```python
from build123d import *

# Parameters (mm, degrees)
PLATE_OUTLINE_SKETCH_R = 10
BASE_PLATE_30MM_DEPTH  = 30
TOP_POCKET_CUT_DEPTH   = 25


with BuildPart() as part:
    # Plate Outline Sketch → Base Plate 30mm (new body)
    with BuildSketch(Plane(origin=(0, 0, 0), x_dir=(1, 0, 0), z_dir=(0, 1, 0))):
        with BuildLine():
            Line((-90, -88), (-90, -17.408786158))
            ThreePointArc((-90, -17.408786158), (-85.756556041, -5.090874739), (-74.826905826, 2))
            Line((-74.826905826, 2), (-4.826905826, 19.408786158))
            ThreePointArc((-4.826905826, 19.408786158), (0, 20), (4.826905826, 19.408786158))
            Line((4.826905826, 19.408786158), (74.826905826, 2))
            ThreePointArc((74.826905826, 2), (85.756556041, -5.090874739), (90, -17.408786158))
            Line((90, -17.408786158), (90, -88))
            ThreePointArc((90, -88), (78.164965809, -106.257418584), (56.666666667, -102.90711985))
            ThreePointArc((56.666666667, -102.90711985), (0, -81.262379212), (-56.666666667, -102.90711985))
            ThreePointArc((-56.666666667, -102.90711985), (-78.164965809, -106.257418584), (-90, -88))
        make_face()
        with Locations(Location((0, 0, 0), (0, 0, 270))):
            Circle(PLATE_OUTLINE_SKETCH_R, mode=Mode.SUBTRACT)
        with Locations(Location((-70, -88, 0), (0, 0, 270))):
            Circle(PLATE_OUTLINE_SKETCH_R, mode=Mode.SUBTRACT)
        with Locations(Location((70, -88, 0), (0, 0, 90))):
            Circle(PLATE_OUTLINE_SKETCH_R, mode=Mode.SUBTRACT)
        with BuildLine():
            Line((-80, -68.635083269), (-80, -17.408786158))
            ThreePointArc((-80, -17.408786158), (-75.428711332, -4.682637227), (-63.804513336, 2.226021665))
            Line((-63.804513336, 2.226021665), (-20.095749168, 10.695194253))
            ThreePointArc((-20.095749168, 10.695194253), (-15.433233379, 9.136955423), (-14.358465626, 4.339869223))
            ThreePointArc((-14.358465626, 4.339869223), (0, -15), (14.358465626, 4.339869223))
            ThreePointArc((14.358465626, 4.339869223), (15.433233379, 9.136955423), (20.095749168, 10.695194253))
            Line((20.095749168, 10.695194253), (63.804513336, 2.226021665))
            ThreePointArc((63.804513336, 2.226021665), (75.428711332, -4.682637227), (80, -17.408786158))
            Line((80, -17.408786158), (80, -68.635083269))
            ThreePointArc((80, -68.635083269), (78.061862178, -72.587930344), (73.75, -73.476312452))
            ThreePointArc((73.75, -73.476312452), (60.955053625, -76.033841674), (55.004181334, -87.645849573))
            ThreePointArc((55.004181334, -87.645849573), (52.221345421, -92.010026772), (47.064070693, -91.571010006))
            ThreePointArc((47.064070693, -91.571010006), (0, -76.262379212), (-47.064070693, -91.571010006))
            ThreePointArc((-47.064070693, -91.571010006), (-52.221345421, -92.010026772), (-55.004181334, -87.645849573))
            ThreePointArc((-55.004181334, -87.645849573), (-60.955053625, -76.033841674), (-73.75, -73.476312452))
            ThreePointArc((-73.75, -73.476312452), (-78.061862178, -72.587930344), (-80, -68.635083269))
        make_face(mode=Mode.SUBTRACT)
    extrude(amount=BASE_PLATE_30MM_DEPTH)

    # Top Pocket Sketch → Top Pocket Cut (add)
    with BuildSketch(Plane.XZ):
        with BuildLine():
            Line((-20.095749168, -10.695194253), (-63.804513336, -2.226021665))
            ThreePointArc((-63.804513336, -2.226021665), (-75.428711332, 4.682637227), (-80, 17.408786158))
            Line((-80, 17.408786158), (-80, 68.635083269))
            ThreePointArc((-80, 68.635083269), (-78.061862178, 72.587930344), (-73.75, 73.476312452))
            ThreePointArc((-73.75, 73.476312452), (-60.955053625, 76.033841674), (-55.004181334, 87.645849573))
            ThreePointArc((-55.004181334, 87.645849573), (-52.221345421, 92.010026772), (-47.064070693, 91.571010006))
            ThreePointArc((-47.064070693, 91.571010006), (0, 76.262379212), (47.064070693, 91.571010006))
            ThreePointArc((47.064070693, 91.571010006), (52.221345421, 92.010026772), (55.004181334, 87.645849573))
            ThreePointArc((55.004181334, 87.645849573), (60.955053625, 76.033841674), (73.75, 73.476312452))
            ThreePointArc((73.75, 73.476312452), (78.061862178, 72.587930344), (80, 68.635083269))
            Line((80, 68.635083269), (80, 17.408786158))
            ThreePointArc((80, 17.408786158), (75.428711332, 4.682637227), (63.804513336, -2.226021665))
            Line((63.804513336, -2.226021665), (20.095749168, -10.695194253))
            ThreePointArc((20.095749168, -10.695194253), (15.433233379, -9.136955423), (14.358465626, -4.339869223))
            ThreePointArc((14.358465626, -4.339869223), (0, 15), (-14.358465626, -4.339869223))
            ThreePointArc((-14.358465626, -4.339869223), (-15.433233379, -9.136955423), (-20.095749168, -10.695194253))
        make_face()
    extrude(amount=-TOP_POCKET_CUT_DEPTH)


solid = part.part
```
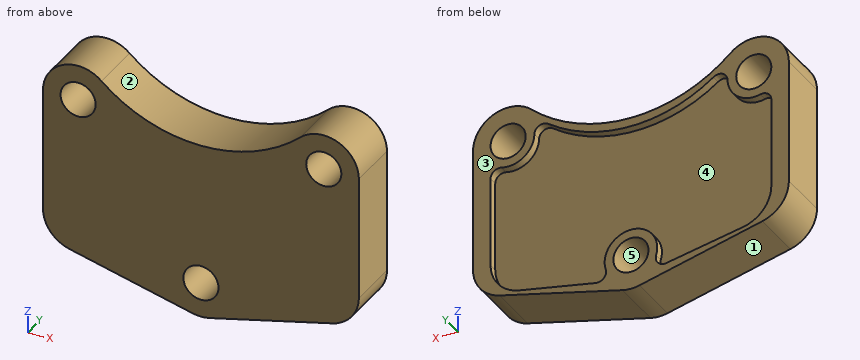
Verification items for the finished model (mm, model axes). Face numbers are marked on the shaded views. A direction names the side the tool comes from. Round coordinates to 2 decimals unless told otherwise and drop trailing zeros. Write each loop counter-clockwise with the first axis right and the second up, starting at its lowest first coordinate (ties: lowest second). Pieces come first, ordered by that corner, then holes.
1. Scan lines: L1, parallel to X at y = 27.5, z = 33; L2, parallel to X at y = 12, z = 88; L3, parallel to Y at x = -14, z = 53. Record each from-to range of solid material in increasing order.
2. Gauge pin test, flat ends, axial feed: P1, Ø16, axis at x = -70, z = 88, coming from the -Y side; P2, Ø3, axis at x = -3.5, y = 14.5, coming from the -Z side; P3, Ø1.5, axis at x = -19.5, y = 5, coming from the +Z side; P4, Ø6, axis at x = 60, z = 33.5, coming from the +Y side. Record the tip position at first contact, or that the pin passes through.
3. Section check C-C on z = 0. Enter the section's corners in (x, y), plus the area to 3 significant figures.
4. Access from +Z, -Z, +X, -X, +Y, -Y to the whole of each face (thin tool, end or side, straight path). Record for the marked faces 4 and 5.
5. Draft check along X on the marked faces 1, 2 and 3. Enter one of: +X half, -X half, draft (parallel to the pull), parting line (faces both ways), or undercut.
6. Section check A-A on x = 0. Enter the section's corners in (y, z).
7. Section check B-B on y = 11.5. Enter the section's corners in (x, z).
8. Section check D-D on x = -70. Enter the section's corners in (y, z), plus the area to 3 significant figures.
Answer:
1. L1: x = -90 to -80, 80 to 90
1. L2: x = -90 to -80, -60 to -33.17, 33.17 to 60, 80 to 90
1. L3: y = 0 to 25
2. P1: passes through
2. P2: stops at z = -19.9
2. P3: stops at z = 83.71
2. P4: stops at y = 25
3. outline: (-79.85, 0) - (-10, 0) - (-10, 30) - (-15, 30) - (-15, 25) - (-69.85, 25) - (-69.85, 30) - (-79.85, 30) - close; (10, 0) - (79.85, 0) - (79.85, 30) - (69.85, 30) - (69.85, 25) - (15, 25) - (15, 30) - (10, 30) - close
3. area: 3,640 mm2
4. face 4: +Y
4. face 5: +Y, -Y
5. face 1: -X half
5. face 2: undercut
5. face 3: draft
6. outline: (0, -20) - (30, -20) - (30, -10) - (0, -10) - close; (0, 10) - (30, 10) - (30, 15) - (25, 15) - (25, 76.26) - (30, 76.26) - (30, 81.26) - (0, 81.26) - close
7. outline: (-90, 17.41) arc R20 ccw to (-74.83, -2) - (-4.83, -19.41) arc R20 ccw to (4.83, -19.41) - (74.83, -2) arc R20 ccw to (90, 17.41) - (90, 88) arc R20 ccw to (56.67, 102.91) arc R85 cw to (-56.67, 102.91) arc R20 ccw to (-90, 88) - close; hole circle Ø20 at (-70, 88); hole circle Ø20 at (0, 0); hole circle Ø20 at (70, 88)
8. outline: (0, -3.2) - (30, -3.2) - (30, 0.09) - (25, 0.09) - (25, 73) - (30, 73) - (30, 78) - (0, 78) - close; (0, 98) - (30, 98) - (30, 108) - (0, 108) - close
8. area: 2,370 mm2
